```python
from build123d import *

# Parameters (mm, degrees)
SKETCH1_R           = 30
BOSS_EXTRUDE1_DEPTH = 10
SKETCH2_W           = 58.621984262
SKETCH2_H           = 13
CUT_EXTRUDE1_DEPTH  = 33
SKETCH3_R           = 6.5
CUT_EXTRUDE2_DEPTH  = 33
CHAMFER1_SIZE       = 1.67


with BuildPart() as part:
    # Sketch1 → Boss-Extrude1 (new body)
    with BuildSketch(Plane(origin=(0, 0, 0), x_dir=(1, 0, 0), z_dir=(0, 1, 0))):
        with Locations(Location((0, 0, 0), (0, 0, 270))):
            Circle(SKETCH1_R)
    extrude(amount=BOSS_EXTRUDE1_DEPTH)

    # Sketch2 → Cut-Extrude1 (cut)
    with BuildSketch(Plane(origin=(0, 10, 0), x_dir=(1, 0, 0), z_dir=(0, 1, 0))):
        with Locations((30, 0)):
            Rectangle(SKETCH2_W, SKETCH2_H)
    extrude(amount=-CUT_EXTRUDE1_DEPTH, mode=Mode.SUBTRACT)

    # Sketch3 → Cut-Extrude2 (cut)
    with BuildSketch(Plane(origin=(0, 10, 0), x_dir=(1, 0, 0), z_dir=(0, 1, 0))):
        Circle(SKETCH3_R)
    extrude(amount=-CUT_EXTRUDE2_DEPTH, mode=Mode.SUBTRACT)

    # Chamfer1
    chamfer1_edges = [part.edges().sort_by_distance(p)[0] for p in [
        (-30, 0, 0),
        (-30, 10, 0),
    ]]
    chamfer(chamfer1_edges, length=CHAMFER1_SIZE)


solid = part.part
```
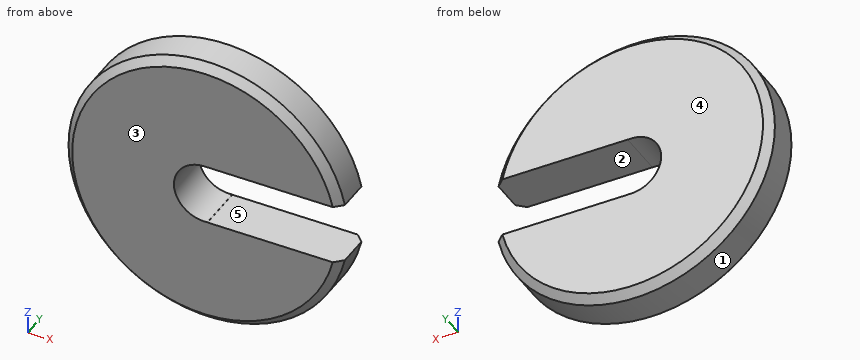
Model file for the job. Use its own axes, mm. Face numbers are marked on the shaded views. A direction names the side the tool comes from. Give positions to 0.01 mm unless a question says otherwise; leave off trailing zeros. Order: outer loops, then holes, each group sorted by start corner. A loop starts at its lowest first (then second) coordinate and runs counter-clockwise, first axis right, second up.
1) 3-axis set-ups, long thin cutter, end or side, ignore diameter. For the marked faces 4 and 5: which of +Z, -Z, +X, -X, +Y, -Y reach the whole face in a straight line?
2) Wall check: probe 1 along X at (y, z) = (5.25, 0); probe 2 along Z at (x, y) = (21.5, 6.25); probe 3 along Z at (x, y) = (25, 2). Give the ranges that are in metal, low to high.
3) Saw through at A-A, the plane x = 0. Write the cut outline in (y, z).
4) Pin check, flat tips, straight feed: pin 1 (10 mm diameter, centred on x = 1.5, z = -22.5, fed in from -Y); pin 2 (1 mm diameter, centred on x = 21.5, y = 3, fed in from -Z); pin 3 (6 mm diameter, centred on y = 5.5, z = -0.5, fed in from -X); pin 4 (3 mm diameter, centred on x = 21, y = 2, fed in from +Z). Stop position of each tip, or through.
5) Mould opens along Z. For the marked faces 1, 2 and 3 say: +Z half, -Z half, draft (parallel to the pull), parting line (faces both ways), or undercut.
6) Saw through at C-C, the plane z = 0. Write the cut outline in (x, y).
Computed:
1. face 4: +Z, -Z, +X, -X, +Y
1. face 5: +X, +Y, -Y
2. probe 1: x = -30 to -6.5
2. probe 2: z = -20.92 to -6.5, 6.5 to 20.92
2. probe 3: z = -16.58 to -6.5, 6.5 to 16.58
3. outline: (0, -28.33) - (1.67, -30) - (8.33, -30) - (10, -28.33) - (10, -6.5) - (0, -6.5) - close; (0, 6.5) - (10, 6.5) - (10, 28.33) - (8.33, 30) - (1.67, 30) - (0, 28.33) - close
4. pin 1: stops at y = 0
4. pin 2: stops at z = -21.42
4. pin 3: stops at x = -30
4. pin 4: stops at z = 22.8
5. face 1: parting line
5. face 2: undercut
5. face 3: draft
6. outline: (-30, 1.67) - (-28.33, 0) - (-6.5, 0) - (-6.5, 10) - (-28.33, 10) - (-30, 8.33) - close
